Design review of the part built by this model. Coordinates are the model's own, in mm. Coordinates: 2 decimals unless noted, no trailing zeros. Order: outer loops, then holes, each group sorted by start corner. A loop starts at its lowest first (then second) coordinate and runs counter-clockwise, first axis right, second up. Notation, with made-up numbers: M 8,34 L 15,34 A17 cw 15,38 Z; hole C 82.5,27 d2. An arc over 180 degrees is marked long. Use CSV: the item, a comma, the result in double quotes.
```python
from build123d import *

# Parameters (mm, degrees)
SKETCH1_W           = 30
SKETCH1_H           = 1070
SKETCH2_R           = 10
BOSS_EXTRUDE1_DEPTH = 6
BOSS_EXTRUDE2_DEPTH = 15
BOSS_EXTRUDE3_START = 13
SKETCH4_R           = 10
BOSS_EXTRUDE3_DEPTH = 13
SKETCH5_R           = 6
BOSS_EXTRUDE4_DEPTH = 7
CHAMFER1_SIZE       = 1


with BuildPart() as part:
    # Sketch1 → Revolve1 (revolve)
    with BuildSketch(Plane.XZ, mode=Mode.PRIVATE) as revolve1_sk:
        with Locations((15, 0)):
            Rectangle(SKETCH1_W, SKETCH1_H)
    revolve(revolve1_sk.sketch.rotate(Axis((0, 0, 535), (0, 0, -1)), 180), axis=Axis((0, 0, 535), (0, 0, -1)))

    # Sketch2 → Boss-Extrude1 (add)
    with BuildSketch(Plane(origin=(0, 0, -535), x_dir=(-1, 0, 0), z_dir=(0, 0, -1))):
        Circle(SKETCH2_R)
    extrude(amount=BOSS_EXTRUDE1_DEPTH)

    # Sketch3 → Boss-Extrude2 (add)
    with BuildSketch(Plane(origin=(0, 0, -541), x_dir=(-1, 0, 0), z_dir=(0, 0, -1))):
        with BuildLine():
            Line((-4.5, 6), (4.5, 6))
            ThreePointArc((4.5, 6), (7.5, 0), (4.5, -6))
            Line((4.5, -6), (-4.5, -6))
            ThreePointArc((-4.5, -6), (-7.5, 0), (-4.5, 6))
        make_face()
    extrude(amount=BOSS_EXTRUDE2_DEPTH)

    # Sketch4 → Boss-Extrude3 (add)
    with BuildSketch(Plane.XY.offset(535).offset(BOSS_EXTRUDE3_START)):
        with Locations(Location((0, 0, 0), (0, 0, 180))):
            Circle(SKETCH4_R)
    extrude(amount=-BOSS_EXTRUDE3_DEPTH)

    # Sketch5 → Boss-Extrude4 (add)
    with BuildSketch(Plane.XY.offset(548)):
        with Locations(Location((0, 0, 0), (0, 0, 180))):
            Circle(SKETCH5_R)
    extrude(amount=BOSS_EXTRUDE4_DEPTH)

    # Chamfer1
    chamfer1_edges = [part.edges().sort_by_distance(p)[0] for p in [
        (7.5, 0, -556),
        (0, -6, -556),
        (-7.5, 0, -556),
        (0, 6, -556),
        (6, 0, 555),
    ]]
    chamfer(chamfer1_edges, length=CHAMFER1_SIZE)


solid = part.part
```
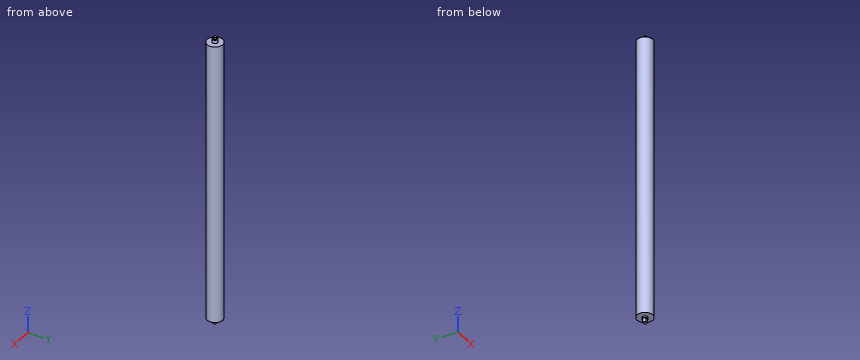
(1) Add section A-A on z = 331.5. State the section outline as (x, y) points, and give its area (3 significant figures).
The answers:
outline,"C 0,0 d60"
area,"2,830 mm2"
(2) Clearance check with flat-ended pins moving along their axes: P1, Ø10, axis at x = -15, y = -8.5, coming from the +Z side; P2, Ø1, axis at x = 6.5, z = 164, coming from the +Y side; P3, Ø3, axis at y = 20.5, z = -442, coming from the +X side; P4, Ø10, axis at x = 2.5, y = 4.5, coming from the +Z side. State where each tip first meets the part, or that it passes through.
The answers:
P1,"stops at z = 535"
P2,"stops at y = 29.39"
P3,"stops at x = 23.22"
P4,"stops at z = 555"
(3) Add section B-B on x = 20. State the section outline as (y, z) points, and give its area (3 significant figures).
The answers:
outline,"M -22.36,-535 L 22.36,-535 L 22.36,535 L -22.36,535 Z"
area,"47,900 mm2"
(4) Wall thickness on probe 1 along Z at (x, y) = (-13.5, 0); probe 2 along X at (y, z) = (-3, 335): over which ranges is each line inside the solid? List them lowest first.
The answers:
probe 1,"z = -535 to 535"
probe 2,"x = -29.85 to 29.85"
